Input: dimensioned drawing with shaded views. Units: mm. Origin: part minimum x, y, z. A direction names the side the tool comes from. Give positions to 0.01 mm unless a question says otherwise; leave off trailing zeros. Loops run counter-clockwise (first coordinate to the right, second up) from the corner with the lowest first, then second, coordinate; pieces in that order, holes last. Notation, with made-up numbers: (10.25, -17) -> (62.25, -17) arc R33 ccw to (62.25, 14) -> close; hole circle Ø8 at (20.25, 72). An arc over 180 degrees is marked (long way). One line per question, with ' | ' between items. Start each with the question number.
Item 1: Section C-C on x = 12.5. Return loops of the section in (y, z).
Item 2: Pin query (flat end, axial travel): P1, Ø1.5, axis at x = 33.5, z = 6, coming from the +Y side; P2, Ø4, axis at x = 59, z = 5, coming from the -Y side; P3, Ø1, axis at x = 24, z = 7.5, coming from the +Y side. Return the tip coordinate at first contact, or that it passes through.
Item 3: Section D-D on x = 67. Return loops of the section in (y, z), then the cut area to 3 significant figures.
Item 4: Section A-A on y = 6. Return loops of the section in (x, z).
Item 5: Material intervals for line 1 along Y through (x, z) = (70, 5.75); line 2 along X through (y, z) = (5, 8.5); line 3 along X through (y, z) = (11.25, 6), sorted ascending. Write a range as [from, to].
Item 6: Set-up query: the marked faces 1 and 2. Return all of +Z, -Z, +X, -X, +Y, -Y with unobstructed straight access to the full face (end or side cutting, diameter ignored); none if empty.
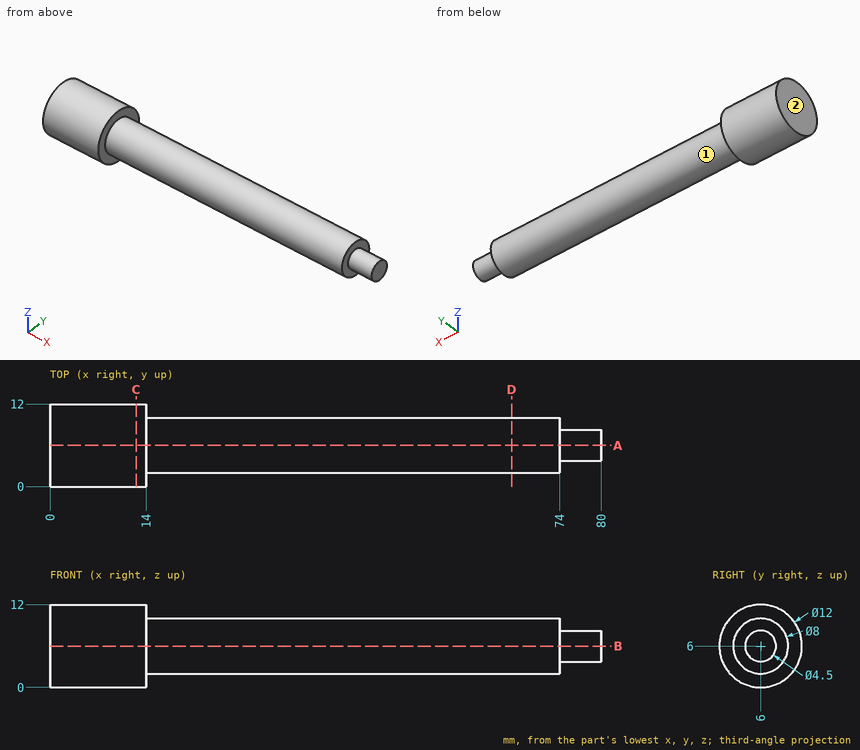
Result sheet:
1) outline: circle Ø12 at (6, 6)
2) P1: stops at y = 10 | P2: stops at y = 2 | P3: stops at y = 9.87
3) outline: circle Ø8 at (6, 6) | area: 50.3 mm²
4) outline: (0, 0) -> (14, 0) -> (14, 2) -> (74, 2) -> (74, 3.75) -> (80, 3.75) -> (80, 8.25) -> (74, 8.25) -> (74, 10) -> (14, 10) -> (14, 12) -> (0, 12) -> close
5) line 1: y = [2.01, 9.99] | line 2: x = [0, 74] | line 3: x = [0, 14]
6) face 1: +X | face 2: +Z, -Z, -X, +Y, -Y
